The listing builds one solid part. Answer for the finished solid, in the listing's coordinates (mm). A direction names the side the tool comes from. Round coordinates to 2 decimals unless told otherwise and drop trailing zeros. Write each loop counter-clockwise with the first axis right and the second up, starting at its lowest first coordinate (ties: lowest second). Pieces come first, ordered by that corner, then holes. Notation, with made-up numbers: (86.25, 48) - (116.25, 48) arc R19 cw to (116.25, 73) - close; hole circle Ø6 at (-3.5, 31.5). An arc over 180 degrees is marked (long way). Return JSON: item names as keys, results as strings. Group by question number.
(1) Determine the mould class of faces 4 (the flat face through (-5, 6.5, -2)), 5 (the cylindrical face through (-4.88, 0.25, 1.08)), 6 (the flat face through (-10, 0, 2)), 7 (the cylindrical face through (-10.74, 3.45, -2.38)) for opening direction Z: +Z half, -Z half, draft (parallel to the pull), parting line (faces both ways), or undercut.
(2) Section D-D, the plane x = 4.5 is taken. Write down the section's boundary in (y, z).
(3) Each of these flat-tipped pins is pushed along its axis until it touches: pin 1 (4 mm diameter, centred on x = -3, y = 5, fed in from +Z); pin 2 (1.5 mm diameter, centred on y = 2, z = -7.5, fed in from -X); pin 3 (1.5 mm diameter, centred on x = -5, y = 5, fed in from +Z). Where does it stop, or does it pass through?
(4) Section B-B, the plane y = 3.5 is taken. Write down the section's boundary in (x, z).
(5) Which of the six approach directions +Z, -Z, +X, -X, +Y, -Y give full straight-line access (tool end or side, diameter ignored) to faces 1 (the cylindrical face through (4.88, 6.75, 1.08)), 2 (the flat face through (5, 0.5, -2)), 3 (the cylindrical face through (-3.905, 3.451, -0.867))?
(6) Section A-A, the plane x = 0 is taken. Write down the section's boundary in (y, z), then the cut area to 3 significant figures.
(7) Section C-C, the plane z = 0.75 is taken. Write down the section's boundary in (x, y).
(8) Find the intervals of material crossed by line 1 along X through (y, z) = (0.15, 0); line 2 along Y through (x, z) = (4.5, 7.25); line 3 along X through (y, z) = (6.75, -2.25), in increasing order. Write a range as [from, to].
```python
from build123d import *

# Parameters (mm, degrees)
SKETCH1_R           = 11
SKETCH1_R_2         = 4
BOSS_EXTRUDE1_DEPTH = 7
SKETCH2_R           = 10
SKETCH2_R_2         = 5
CUT_EXTRUDE1_DEPTH  = 0.5
CUT_EXTRUDE2_START  = -0.5
SKETCH3_R           = 10
SKETCH3_R_2         = 5
CUT_EXTRUDE2_DEPTH  = 0.5


with BuildPart() as part:
    # Sketch1 → Boss-Extrude1 (new body)
    with BuildSketch(Plane(origin=(0, 0, 0), x_dir=(1, 0, 0), z_dir=(0, 1, 0))):
        with Locations(Location((0, 0, 0), (0, 0, 270))):
            Circle(SKETCH1_R)
        with Locations(Location((0, 0, 0), (0, 0, 270))):
            Circle(SKETCH1_R_2, mode=Mode.SUBTRACT)
    extrude(amount=BOSS_EXTRUDE1_DEPTH)

    # Sketch2 → Cut-Extrude1 (cut)
    with BuildSketch(Plane.XZ):
        with Locations(Location((0, 0, 0), (0, 0, 270))):
            Circle(SKETCH2_R)
        with Locations(Location((0, 0, 0), (0, 0, 270))):
            Circle(SKETCH2_R_2, mode=Mode.SUBTRACT)
    extrude(amount=-CUT_EXTRUDE1_DEPTH, mode=Mode.SUBTRACT)

    # Sketch3 → Cut-Extrude2 (cut)
    with BuildSketch(Plane(origin=(0, 7, 0), x_dir=(1, 0, 0), z_dir=(0, 1, 0)).offset(CUT_EXTRUDE2_START)):
        with Locations(Location((0, 0, 0), (0, 0, 90))):
            Circle(SKETCH3_R)
        with Locations(Location((0, 0, 0), (0, 0, 90))):
            Circle(SKETCH3_R_2, mode=Mode.SUBTRACT)
    extrude(amount=CUT_EXTRUDE2_DEPTH, mode=Mode.SUBTRACT)


solid = part.part
```
Working result:
{
 "1": {"face 4": "undercut", "face 5": "undercut", "face 6": "draft", "face 7": "parting line"},
 "2": {"outline": "(0, -10.04) - (7, -10.04) - (7, -8.93) - (6.5, -8.93) - (6.5, -2.18) - (7, -2.18) - (7, 2.18) - (6.5, 2.18) - (6.5, 8.93) - (7, 8.93) - (7, 10.04) - (0, 10.04) - (0, 8.93) - (0.5, 8.93) - (0.5, 2.18) - (0, 2.18) - (0, -2.18) - (0.5, -2.18) - (0.5, -8.93) - (0, -8.93) - close"},
 "3": {"pin 1": "stops at z = 10.95", "pin 2": "stops at x = -8.69", "pin 3": "stops at z = 10.15"},
 "4": {"outline": "circle Ø22 at (0, 0); hole circle Ø8 at (0, 0)"},
 "5": {"face 1": "+Y", "face 2": "-Y", "face 3": "+Y, -Y"},
 "6": {"outline": "(0, -11) - (7, -11) - (7, -10) - (6.5, -10) - (6.5, -5) - (7, -5) - (7, -4) - (0, -4) - (0, -5) - (0.5, -5) - (0.5, -10) - (0, -10) - close; (0, 4) - (7, 4) - (7, 5) - (6.5, 5) - (6.5, 10) - (7, 10) - (7, 11) - (0, 11) - (0, 10) - (0.5, 10) - (0.5, 5) - (0, 5) - close", "area": "88.0 mm^2"},
 "7": {"outline": "(-10.97, 0) - (-9.97, 0) - (-9.97, 0.5) - (-4.94, 0.5) - (-4.94, 0) - (-3.93, 0) - (-3.93, 7) - (-4.94, 7) - (-4.94, 6.5) - (-9.97, 6.5) - (-9.97, 7) - (-10.97, 7) - close; (3.93, 0) - (4.94, 0) - (4.94, 0.5) - (9.97, 0.5) - (9.97, 0) - (10.97, 0) - (10.97, 7) - (9.97, 7) - (9.97, 6.5) - (4.94, 6.5) - (4.94, 7) - (3.93, 7) - close"},
 "8": {"line 1": "x = [-11, -10], [-5, -4], [4, 5], [10, 11]", "line 2": "y = [0.5, 6.5]", "line 3": "x = [-10.77, -9.74], [-4.47, -3.31], [3.31, 4.47], [9.74, 10.77]"}
}
